```python
from build123d import *

# Parameters (mm, degrees)
SKETCH1_W             = 10
SKETCH1_H             = 17
BOSS_EXTRUDE1_DEPTH   = 2
SKETCH2_W             = 14
SKETCH2_H             = 10
BOSS_EXTRUDE2_DEPTH   = 2
SKETCH3_R             = 1.4
CUT_EXTRUDE1_DEPTH    = 10
CHAMFER1_SIZE         = 1
M2_TAPPED_HOLE1_D     = 1.6
M2_TAPPED_HOLE1_DEPTH = 5.2
M2_TAPPED_HOLE1_TIP   = 0.480688495


with BuildPart() as part:
    # Sketch1 → Boss-Extrude1 (new body)
    with BuildSketch(Plane(origin=(0, 0, 0), x_dir=(1, 0, 0), z_dir=(0, 1, 0))):
        with Locations((5, 8.5)):
            Rectangle(SKETCH1_W, SKETCH1_H)
    extrude(amount=BOSS_EXTRUDE1_DEPTH)

    # Sketch2 → Boss-Extrude2 (add)
    with BuildSketch(Plane(origin=(0, 2, 0), x_dir=(1, 0, 0), z_dir=(0, 1, 0))):
        with Locations((17, 12)):
            Rectangle(SKETCH2_W, SKETCH2_H)
    extrude(amount=-BOSS_EXTRUDE2_DEPTH)

    # Sketch3 → Cut-Extrude1 (cut)
    with BuildSketch(Plane(origin=(0, 2, 0), x_dir=(1, 0, 0), z_dir=(0, 1, 0))):
        with Locations(Location((21, 12, 0), (0, 0, 270))):
            Circle(SKETCH3_R)
        with Locations(Location((13, 12, 0), (0, 0, 270))):
            Circle(SKETCH3_R)
    extrude(amount=-CUT_EXTRUDE1_DEPTH, mode=Mode.SUBTRACT)

    # Chamfer1
    chamfer1_edges = [part.edges().sort_by_distance(p)[0] for p in [
        (0, 1, -17),
        (0, 1, 0),
        (10, 1, 0),
        (24, 1, -17),
        (24, 1, -7),
    ]]
    chamfer(chamfer1_edges, length=CHAMFER1_SIZE)

    # M2 Tapped Hole1
    with Locations(Plane(origin=(0, 2, 0), x_dir=(1, 0, 0), z_dir=(0, 1, 0))):
        with Locations((8, 10.7), (8, 2.7)):
            Hole(M2_TAPPED_HOLE1_D / 2, depth=M2_TAPPED_HOLE1_DEPTH)
            with Locations((0, 0, -(M2_TAPPED_HOLE1_DEPTH + M2_TAPPED_HOLE1_TIP / 2))):  # 118° drill point
                Cone(0, M2_TAPPED_HOLE1_D / 2, M2_TAPPED_HOLE1_TIP, mode=Mode.SUBTRACT)


solid = part.part
```
Geometry check sheet. Reference: the model listing, model coordinates, mm. A direction names the side the tool comes from. Coordinates: 2 decimals unless noted, no trailing zeros. Loops run counter-clockwise (first coordinate to the right, second up) from the corner with the lowest first, then second, coordinate; pieces in that order, holes last.
Item 1: Sectioned sample at C-C, the plane z = -12. Record the boundary of the cut face in (x, y).
Item 2: Access from +Z, -Z, +X, -X, +Y, -Y to the whole of each face (thin tool, end or side, straight path). Record for faces 5 (the face through (5, 1, 0)), 6 (the face through (16, 1, -7)).
Item 3: Go/stop test with flat-tipped pins: pin 1 Ø2.5 at (x, z) = (8, -2.7) entering from -Y; pin 2 Ø1 at (x, y) = (15.5, 1) entering from +Z. Record where each tip stops, or that it passes through.
Item 4: Sectioned sample at D-D, the plane y = 0.85. Record the boundary of the cut face in (x, z).
Item 5: Release check for a two-part mould opening along Z. For faces 1 (the face through (0.5, 1, -0.5)), 2 (the face through (23.5, 1, -16.5)), 3 (the face through (0, 1, -8)), 4 (the face through (8.63, 0.99, -10.21)) record: released by +Z, released by -Z, zero draft, split by the parting line, or undercut.
Item 6: Sectioned sample at A-A, the plane z = -2.7. Record the boundary of the cut face in (x, y), then the cut area to 3 significant figures.
Item 7: Sectioned sample at B-B, the plane x = 21. Record the boundary of the cut face in (y, z).
Item 8: Thickness scan on line 1 (X direction, y = 1, z = -12); line 2 (Z direction, x = 8, y = 0.6); line 3 (X direction, y = 0.8, z = -2.7). Record the ranges inside material, lowest first.
Check result:
1. outline: (0, 0) - (11.6, 0) - (11.6, 2) - (0, 2) - close; (14.4, 0) - (19.6, 0) - (19.6, 2) - (14.4, 2) - close; (22.4, 0) - (24, 0) - (24, 2) - (22.4, 2) - close
2. face 5: +Z, +X, -X, +Y, -Y
2. face 6: +Z, +X, +Y, -Y
3. pin 1: stops at y = 0
3. pin 2: stops at z = -7
4. outline: (0, -16) - (1, -17) - (23, -17) - (24, -16) - (24, -8) - (23, -7) - (10, -7) - (10, -1) - (9, 0) - (1, 0) - (0, -1) - close; hole circle Ø1.6 at (8, -10.7); hole circle Ø1.6 at (8, -2.7); hole circle Ø2.8 at (13, -12); hole circle Ø2.8 at (21, -12)
5. face 1: released by +Z
5. face 2: released by -Z
5. face 3: zero draft
5. face 4: undercut
6. outline: (0, 0) - (7.2, 0) - (7.2, 2) - (0, 2) - close; (8.8, 0) - (10, 0) - (10, 2) - (8.8, 2) - close
6. area: 16.8 mm2
7. outline: (0, -17) - (2, -17) - (2, -13.4) - (0, -13.4) - close; (0, -10.6) - (2, -10.6) - (2, -7) - (0, -7) - close
8. line 1: x = 0 to 11.6, 14.4 to 19.6, 22.4 to 24
8. line 2: z = -17 to -11.5, -9.9 to -3.5, -1.9 to 0
8. line 3: x = 0 to 7.2, 8.8 to 10
